Work out the finished part from the listing and answer in its coordinate system (mm). A direction names the side the tool comes from. Round coordinates to 2 decimals unless told otherwise and drop trailing zeros. Write each loop counter-clockwise with the first axis right and the second up, starting at its lowest first coordinate (ties: lowest second). Pieces come first, ordered by that corner, then holes.
from build123d import *

# Parameters (mm, degrees)
SKETCH_1_W                   = 78
SKETCH_1_H                   = 15
EXTRUDE_1_DEPTH              = 7.5
HOLE_WIZARD_M6_1_D           = 6.6
HOLE_WIZARD_M6_1_CBORE_D     = 11
HOLE_WIZARD_M6_1_CBORE_DEPTH = 6.8
EXTRUDE_3_DEPTH              = 15
SKETCH_2_W                   = 15
SKETCH_2_H                   = 12
EXTRUDE_2_DEPTH              = 14
HOLE_WIZARD_M6_1_2_D         = 5
CUT_EXTRUDE_1_DEPTH          = 51.182168148
CHAMFER_1_SIZE               = 1
FILLET_2_R                   = 10


with BuildPart() as part:
    # 草图1 → 凸台-拉伸1 (new, symmetric)
    with BuildSketch(Plane(origin=(0, 0, 0), x_dir=(1, 0, 0), z_dir=(0, 1, 0))):
        Rectangle(SKETCH_1_W, SKETCH_1_H)
    extrude(amount=EXTRUDE_1_DEPTH, both=True)

    # Hole Wizard M6 _1 (through all)
    with Locations(Plane.XZ.offset(7.5)):
        with Locations((29, 0), (-8, 0)):
            CounterBoreHole(HOLE_WIZARD_M6_1_D / 2, HOLE_WIZARD_M6_1_CBORE_D / 2, HOLE_WIZARD_M6_1_CBORE_DEPTH)

    # 草图8 → 凸台-拉伸3 (add)
    with BuildSketch(Plane(origin=(0, 7.5, 0), x_dir=(1, 0, 0), z_dir=(0, 1, 0))):
        Polygon((-24, 12.5), (-39, 12.5), (-39, 7.5), (-4, 7.5), align=None)
    extrude(amount=-EXTRUDE_3_DEPTH)

    # 草图2 → 凸台-拉伸2 (add)
    with BuildSketch(Plane(origin=(0, -7.5, 0), x_dir=(1, 0, 0), z_dir=(0, 1, 0))):
        with Locations((-31.5, 6.5)):
            Rectangle(SKETCH_2_W, SKETCH_2_H)
    extrude(amount=-EXTRUDE_2_DEPTH)

    # Hole Wizard M6 _1 2 (through all)
    with Locations(Plane(origin=(-28.5, 0, -0.5), x_dir=(1, 0, 0), z_dir=(0, 0, 1))):
        with Locations((-3, -15.5)):
            Hole(HOLE_WIZARD_M6_1_2_D / 2)

    # 草图9 → 切除-拉伸1 (cut, through all)
    with BuildSketch(Plane(origin=(0, -21.5, 0), x_dir=(-1, 0, 0), z_dir=(0, -1, 0))):
        Polygon((39, 0.5), (39, -7.5), (17, -7.5), align=None)
    extrude(amount=-CUT_EXTRUDE_1_DEPTH, mode=Mode.SUBTRACT)

    # 倒角1
    chamfer_1_edges = [part.edges().sort_by_distance(p)[0] for p in [
        (-39, 7.5, -6.5),
        (-39, -21.5, -6.5),
        (-24, -21.5, -6.5),
        (39, 0, 7.5),
        (39, 0, -7.5),
    ]]
    chamfer(chamfer_1_edges, length=CHAMFER_1_SIZE)

    # 圆角2
    fillet_2_edges = [part.edges().sort_by_distance(p)[0] for p in [
        (-4, 0, -7.5),
    ]]
    fillet(fillet_2_edges, radius=FILLET_2_R)


solid = part.part
Q1. The mould has two halves that part along Z. Classify faces 1 (the face through (-4.008, -0.105, -7.577)), 2 (the face through (-39, -7, -6)), 3 (the face through (29, -0.7, -4)): +Z half, -Z half, draft (parallel to the pull), parting line (faces both ways), or undercut.
Q2. Given pin 1 (8.5 mm diameter, centred on x = 29, z = 0, fed in from +Y); pin 2 (4 mm diameter, centred on x = -33.5, y = -15, fed in from +Z); pin 3 (1 mm diameter, centred on y = -9.5, z = -5.5, fed in from +X); pin 4 (9 mm diameter, centred on x = 28, z = 2.5, fed in from -Y), each flat-ended and moving along its own axis, determine where each tip first touches the part or whether it passes through.
Q3. Find section D-D (y = -5.5). Determine the outline of the cut face in (x, z).
Q4. A tool of negligible diameter and unlimited length cuts with its end or side. For faces 4 (the face through (-31.6, -12.8, -0.5)), 5 (the face through (-2.92, -4.15, -2.11)), 6 (the face through (39, 0, 0)), 7 (the face through (-24, -14, -6)), from which of +Z, -Z, +X, -X, +Y, -Y can it reach the whole face along a straight path? Write none if from no direction.
Q5. Find section A-A (y = -15.5). Determine the outline of the cut face in (x, z), plus the area to 3 significant figures.
Q6. Find the intervals of material crossed by L1, parallel to X at y = 4, z = -1; L2, parallel to X at y = 6.75, z = -1.5; L3, parallel to Z at x = 29, y = 2, in increasing order.
Q7. Find section B-B (x = 29). Determine the outline of the cut face in (y, z).
Q8. Find section C-C (z = -2.5). Determine the outline of the cut face in (x, y).
Report:
1. face 1: -Z half
1. face 2: draft
1. face 3: undercut
2. pin 1: stops at y = 7.5
2. pin 2: stops at z = -0.5
2. pin 3: stops at x = -24
2. pin 4: stops at y = -7.5
3. outline: (-39, -12.5) - (-24, -12.5) - (-5.19, -7.8) arc R10 cw to (-2.77, -7.5) - (38, -7.5) - (39, -6.5) - (39, 6.5) - (38, 7.5) - (-17, 7.5) - (-39, -0.5) - close; hole circle Ø11 at (-8, 0); hole circle Ø11 at (29, 0)
4. face 4: +Z, +X, -X, -Y
4. face 5: -Y
4. face 6: +Z, -Z, +X, +Y, -Y
4. face 7: +Z, -Z, +X, -Y
5. outline: (-39, -12.5) - (-34, -12.5) - (-34, -0.5) - (-39, -0.5) - close; (-29, -12.5) - (-24, -12.5) - (-24, -0.5) - (-29, -0.5) - close
5. area: 120 mm2
6. L1: x = -39 to -11.14, -4.86 to 25.86, 32.14 to 39
6. L2: x = -38.75 to -10.94, -5.06 to 26.06, 31.94 to 39
6. L3: z = -7.5 to -3.3, 3.3 to 7.5
7. outline: (-7.5, -7.5) - (7.5, -7.5) - (7.5, -3.3) - (-0.7, -3.3) - (-0.7, -5.5) - (-7.5, -5.5) - close; (-7.5, 5.5) - (-0.7, 5.5) - (-0.7, 3.3) - (7.5, 3.3) - (7.5, 7.5) - (-7.5, 7.5) - close
8. outline: (-39, -20.5) - (-38, -21.5) - (-25, -21.5) - (-24, -20.5) - (-24, -7.5) - (-12.9, -7.5) - (-12.9, -0.7) - (-10.15, -0.7) - (-10.15, 7.5) - (-38, 7.5) - (-39, 6.5) - close; (-5.85, -0.7) - (-3.1, -0.7) - (-3.1, -7.5) - (24.1, -7.5) - (24.1, -0.7) - (26.85, -0.7) - (26.85, 7.5) - (-5.85, 7.5) - close; (31.15, -0.7) - (33.9, -0.7) - (33.9, -7.5) - (39, -7.5) - (39, 7.5) - (31.15, 7.5) - close; hole circle Ø5 at (-31.5, -15.5)
